```python
from build123d import *

# Parameters (mm, degrees)
EXTRUDE_1_DEPTH     = 3
SKETCH_2_W          = 27.052742461
SKETCH_2_H          = 3.381592808
CUT_EXTRUDE_1_DEPTH = 3
SKETCH_3_R          = 12.5
EXTRUDE_2_DEPTH     = 24
EXTRUDE_3_DEPTH     = 2


with BuildPart() as part:
    # 草图1 → 凸台-拉伸1 (new body)
    with BuildSketch(Plane.XY):
        with BuildLine():
            Line((-45, 17), (45, 17))
            ThreePointArc((45, 17), (62, 0), (45, -17))
            Line((45, -17), (-45, -17))
            ThreePointArc((-45, -17), (-62, 0), (-45, 17))
        make_face()
    extrude(amount=EXTRUDE_1_DEPTH)

    # 草图2 → 切除-拉伸1 (cut)
    with BuildSketch(Plane(origin=(0, 0, 0), x_dir=(-1, 0, 0), z_dir=(0, 0, -1))):
        with Locations((-38.163690258, 0)):
            Rectangle(SKETCH_2_W, SKETCH_2_H)
    extrude(amount=-CUT_EXTRUDE_1_DEPTH, mode=Mode.SUBTRACT)

    # 草图3 → 凸台-拉伸2 (add)
    with BuildSketch(Plane.XY.offset(3)):
        with Locations((-45, 0)):
            Circle(SKETCH_3_R)
    extrude(amount=EXTRUDE_2_DEPTH)

    # 草图4 → 凸台-拉伸3 (add)
    with BuildSketch(Plane.XY.offset(27)):
        with BuildLine():
            Line((-57.325166215, 2.083333333), (-49.930066486, 45.833333333))
            ThreePointArc((-49.930066486, 45.833333333), (-45, 50), (-40.069933514, 45.833333333))
            Line((-40.069933514, 45.833333333), (-32.674833785, 2.083333333))
            ThreePointArc((-32.674833785, 2.083333333), (-45, -12.5), (-57.325166215, 2.083333333))
        make_face()
    extrude(amount=EXTRUDE_3_DEPTH)


solid = part.part
```
For this review, take the finished solid that the model builds, in its own axes (mm). A direction names the side the tool comes from. Coordinates: 2 decimals unless noted, no trailing zeros. Write each loop counter-clockwise with the first axis right and the second up, starting at its lowest first coordinate (ties: lowest second). Pieces come first, ordered by that corner, then holes. Notation, with made-up numbers: (-13, 49.5) - (8, 49.5) arc R27 cw to (8, 81.5) - close; hole circle Ø1 at (86.25, 72.25). An arc over 180 degrees is marked (long way). Answer in a Markdown table with one row per item. Add a question column.
Q1. We need section D-D, the plane x = -2. State the section outline as (y, z) points, and give its area (3 significant figures).
Q2. For P1, Ø8, axis at y = 15.5, z = 17.5, coming from the +X side; P2, Ø5, axis at y = 32, z = 23.5, coming from the -X side; P3, Ø1.5, axis at x = 4.5, z = 2, coming from the +Y side; P4, Ø0.9, axis at y = 1, z = 2, coming from the +X side, all flat-tipped, find the tip position at first contact; note any pin that passes through.
Q3. We need section A-A, the plane x = 33.5. State the section outline as (y, z) points.
Q4. We need section B-B, the plane y = 0. State the section outline as (x, z) points, and give its area (3 significant figures).
Q5. We need section C-C, the plane z = 14.5. State the section outline as (x, y) points, and give its area (3 significant figures).
Q6. For probe 1 along Z at (x, y) = (-22, 4.5); probe 2 along Z at (x, y) = (-44.5, 25.5); probe 3 along X at (y, z) = (0, 13), list the stretches that pass through material, from the lowest coordinate up.
Q7. Draft analysis for pull direction Y (two halves, no side actions). For faces 1 (the flat face through (38, -1.691, 1)), 2 (the cylindrical face through (-45, 50, 28)), 3 (the flat face through (38, 1.691, 1)), 4 (the flat face through (-45, 26, 27)), state which applies: +Y half, -Y half, draft (parallel to the pull), parting line (faces both ways), or undercut.
Q8. Tool access review of faces 5 (the flat face through (-36.424, 24.265, 27.986)), 6 (the flat face through (-45, 12, 29)), 7 (the flat face through (51.69, 0, 1)), 8 (the cylindrical face through (-62, 0, 1)), 9 (the flat face through (-53.68, 23.65, 27.99)): name each direction out of +Z, -Z, +X, -X, +Y, -Y from which nothing blocks a thin tool from reaching the whole face with its end or side.
Answer list:
| question | item | result |
|---|---|---|
| 1 | outline | (-17, 0) - (17, 0) - (17, 3) - (-17, 3) - close |
| 1 | area | 102 mm2 |
| 2 | P1 | stops at x = -40.1 |
| 2 | P2 | passes through |
| 2 | P3 | stops at y = 17 |
| 2 | P4 | stops at x = 61.99 |
| 3 | outline | (-17, 0) - (-1.69, 0) - (-1.69, 3) - (-17, 3) - close; (1.69, 0) - (17, 0) - (17, 3) - (1.69, 3) - close |
| 4 | outline | (-62, 0) - (24.64, 0) - (24.64, 3) - (-32.5, 3) - (-32.5, 29) - (-57.5, 29) - (-57.5, 3) - (-62, 3) - close; (51.69, 0) - (62, 0) - (62, 3) - (51.69, 3) - close |
| 4 | area | 941 mm2 |
| 5 | outline | circle Ø25 at (-45, 0) |
| 5 | area | 491 mm2 |
| 6 | probe 1 | z = 0 to 3 |
| 6 | probe 2 | z = 27 to 29 |
| 6 | probe 3 | x = -57.5 to -32.5 |
| 7 | face 1 | undercut |
| 7 | face 2 | +Y half |
| 7 | face 3 | undercut |
| 7 | face 4 | draft |
| 8 | face 5 | +Z, +X, +Y |
| 8 | face 6 | +Z, +X, -X, +Y, -Y |
| 8 | face 7 | +Z, -Z |
| 8 | face 8 | -Z, -X |
| 8 | face 9 | +Z, -X, +Y |
